```python
from build123d import *

# Parameters (mm, degrees)
GBT706_2008_050_5_1_DEPTH = 783.5
CUT_EXTRUDE_1_DEPTH       = 399.080472392
CUT_EXTRUDE_2_REACH       = 399.483


with BuildPart() as part:
    # Sketch1 → Gbt706-2008 热轧等边角钢 050×5(1) (new body)
    with BuildSketch(Plane(origin=(391.75, 0, 0), x_dir=(0, -1, 0), z_dir=(-1, 0, 0))):
        with BuildLine():
            Line((0, 0), (0, 50))
            Line((0, 50), (3.333333333, 50))
            ThreePointArc((3.333333333, 50), (4.511844635, 49.511844635), (5, 48.333333333))
            Line((5, 48.333333333), (5, 10.5))
            ThreePointArc((5, 10.5), (6.610912703, 6.610912703), (10.5, 5))
            Line((10.5, 5), (48.333333333, 5))
            ThreePointArc((48.333333333, 5), (49.511844635, 4.511844635), (50, 3.333333333))
            Line((50, 3.333333333), (50, 0))
            Line((50, 0), (0, 0))
        make_face()
    extrude(amount=GBT706_2008_050_5_1_DEPTH)

    # 草图2 → 切除-拉伸1 (cut, through all)
    with BuildSketch(Plane(origin=(0, 0, 0), x_dir=(1, 0, 0), z_dir=(0, 1, 0))):
        Polygon((-335.25, 0), (-335.25, -7.501394609), (-339.727357684, -7.501394609), (-382.795284633, -12.028016136), (-391.75, -21.973235089), (-391.75, -52.501394609), (-406.75, -52.501394609), (-406.75, 7.498605391), (-335.25, 7.498605391), align=None)
    extrude(amount=-CUT_EXTRUDE_1_DEPTH, mode=Mode.SUBTRACT)

    # 草图3 → 切除-拉伸2 (cut, up to next)
    with BuildSketch(Plane.XY.offset(5), mode=Mode.PRIVATE) as cut_extrude_2_sk1:
        with BuildLine():
            Line((-25.75, -25.5), (-21.75, -25.5))
            ThreePointArc((-21.75, -25.5), (-17.25, -30), (-21.75, -34.5))
            Line((-21.75, -34.5), (-25.75, -34.5))
            ThreePointArc((-25.75, -34.5), (-30.25, -30), (-25.75, -25.5))
        make_face()
    cut_extrude_2_tool1 = extrude(cut_extrude_2_sk1.sketch, amount=-CUT_EXTRUDE_2_REACH, mode=Mode.PRIVATE) & part.part
    # 草图3 → 切除-拉伸2 (cut, up to next)
    with BuildSketch(Plane.XY.offset(5), mode=Mode.PRIVATE) as cut_extrude_2_sk2:
        with BuildLine():
            Line((-311.75, -25.5), (-307.75, -25.5))
            ThreePointArc((-307.75, -25.5), (-303.25, -30), (-307.75, -34.5))
            Line((-307.75, -34.5), (-311.75, -34.5))
            ThreePointArc((-311.75, -34.5), (-316.25, -30), (-311.75, -25.5))
        make_face()
    cut_extrude_2_tool2 = extrude(cut_extrude_2_sk2.sketch, amount=-CUT_EXTRUDE_2_REACH, mode=Mode.PRIVATE) & part.part
    add(cut_extrude_2_tool1.solids().sort_by_distance((-23.75, -30, 5))[0], mode=Mode.SUBTRACT)
    add(cut_extrude_2_tool2.solids().sort_by_distance((-309.75, -30, 5))[0], mode=Mode.SUBTRACT)


solid = part.part
```
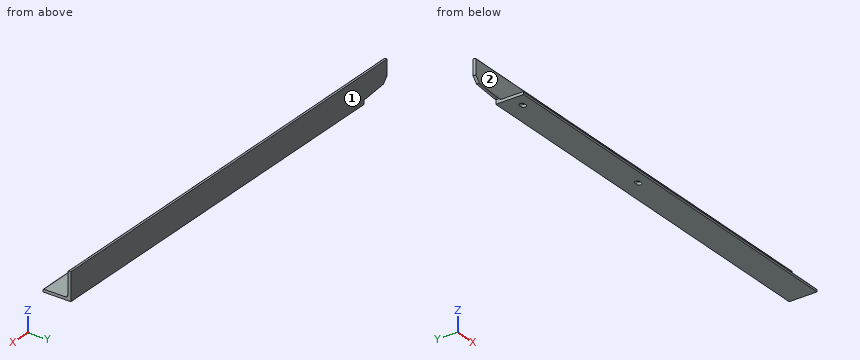
For this review, take the finished solid that the model builds, in its own axes (mm). Face numbers are marked on the shaded views. A direction names the side the tool comes from. Round coordinates to 2 decimals unless told otherwise and drop trailing zeros. Write each loop counter-clockwise with the first axis right and the second up, starting at its lowest first coordinate (ties: lowest second). Pieces come first, ordered by that corner, then holes. Notation, with made-up numbers: (47, 43) - (55, 43) arc R22 cw to (55, 50) - close; hole circle Ø11 at (-13, 28.25). An arc over 180 degrees is marked (long way). Use CSV: the item, a comma, the result in double quotes.
1) For the marked faces 1 and 2, list the 3-axis set-ups (+Z, -Z, +X, -X, +Y, -Y) from which the entire face can be reached by the end or side of a thin tool; tool diameter is ignored.
Conclusion:
face 1,"+Z, -Z, +X, -X, +Y"
face 2,"+Z, +X, -X, -Y"
2) Add section B-B on y = -18. Write out the cut boundary in (x, z), and give its area (4 significant figures).
Conclusion:
outline,"(-335.25, 0) - (391.75, 0) - (391.75, 5) - (-335.25, 5) - close"
area,"3,635 mm^2"
3) Clearance check with flat-ended pins moving along their axes: pin 1 Ø4 at (y, z) = (-29, 3.5) entering from -X; pin 2 Ø1 at (x, z) = (-173, 23) entering from -Y; pin 3 Ø8 at (x, z) = (118.5, 11) entering from -Y. State where each tip first meets the part, or that it passes through.
Conclusion:
pin 1,"stops at x = -335.25"
pin 2,"stops at y = -5"
pin 3,"stops at y = -6.26"
4) Add section A-A on x = 30. Write out the cut boundary in (y, z).
Conclusion:
outline,"(-50, 0) - (0, 0) - (0, 50) - (-3.33, 50) arc R1.67 ccw to (-5, 48.33) - (-5, 10.5) arc R5.5 cw to (-10.5, 5) - (-48.33, 5) arc R1.67 ccw to (-50, 3.33) - close"
5) Wall thickness on line 1 along Y through (x, z) = (258.5, 14); line 2 along Z through (x, y) = (-93, -19.5); line 3 along Z through (x, y) = (151, -3.5): over which ranges is each line inside the solid? List them lowest first. Write a range as from..to.
Conclusion:
line 1,"y = -5..0"
line 2,"z = 0..5"
line 3,"z = 0..49.99"
